from build123d import *

# Parameters (mm, degrees)
BOSS_EXTRUDE1_DEPTH                                 = 17.5
SKETCH2_W                                           = 25
SKETCH2_H                                           = 15
CUT_EXTRUDE1_DEPTH                                  = 47.435439053
M4_TAPPED_HOLE1_D                                   = 3.3
M4_TAPPED_HOLE1_DEPTH                               = 11.5
M4_TAPPED_HOLE1_TIP                                 = 0.991420021
SKETCH5_R                                           = 2
CUT_EXTRUDE2_DEPTH                                  = 56.452682532
FILLET1_R                                           = 2
SKETCH6_R                                           = 4
CUT_EXTRUDE3_DEPTH                                  = 3
CHAMFER1_SIZE                                       = 1
CBORE_FOR_M3_HEX_SOCKET_HEAD_CAP_SCREW1_D           = 3.4
CBORE_FOR_M3_HEX_SOCKET_HEAD_CAP_SCREW1_CBORE_D     = 6.5
CBORE_FOR_M3_HEX_SOCKET_HEAD_CAP_SCREW1_CBORE_DEPTH = 3.4


with BuildPart() as part:
    # Sketch1 → Boss-Extrude1 (new, symmetric)
    with BuildSketch(Plane.XY):
        Polygon((0, 0), (0, 35), (25, 35), (25, 27), (8, 27), (8, 0), align=None)
    extrude(amount=BOSS_EXTRUDE1_DEPTH, both=True)

    # Sketch2 → Cut-Extrude1 (cut, through all)
    with BuildSketch(Plane.ZY):
        with Locations((0, 17.5)):
            Rectangle(SKETCH2_W, SKETCH2_H)
    extrude(amount=-CUT_EXTRUDE1_DEPTH, mode=Mode.SUBTRACT)

    # M4 Tapped Hole1
    with Locations(Plane.ZY):
        with Locations((-12.5, 5), (12.5, 5)):
            Hole(M4_TAPPED_HOLE1_D / 2, depth=M4_TAPPED_HOLE1_DEPTH)
            with Locations((0, 0, -(M4_TAPPED_HOLE1_DEPTH + M4_TAPPED_HOLE1_TIP / 2))):  # 118° drill point
                Cone(0, M4_TAPPED_HOLE1_D / 2, M4_TAPPED_HOLE1_TIP, mode=Mode.SUBTRACT)

    # Sketch5 → Cut-Extrude2 (cut, through all)
    with BuildSketch(Plane.XY.offset(17.5)):
        with Locations((4, 17.5)):
            Circle(SKETCH5_R)
    extrude(amount=-CUT_EXTRUDE2_DEPTH, mode=Mode.SUBTRACT)

    # Fillet1
    fillet1_edges = [part.edges().sort_by_distance(p)[0] for p in [
        (4, 10, -12.5),
        (4, 25, -12.5),
        (4, 25, 12.5),
        (4, 10, 12.5),
    ]]
    fillet(fillet1_edges, radius=FILLET1_R)

    # Sketch6 → Cut-Extrude3 (cut)
    with BuildSketch(Plane.XZ.offset(-27)):
        with Locations((18, 0)):
            Circle(SKETCH6_R)
    extrude(amount=-CUT_EXTRUDE3_DEPTH, mode=Mode.SUBTRACT)

    # Chamfer1
    chamfer1_edges = [part.edges().sort_by_distance(p)[0] for p in [
        (0, 35, 0),
        (8, 27, 0),
        (25, 31, 17.5),
        (4, 0, 17.5),
        (25, 31, -17.5),
        (4, 0, -17.5),
    ]]
    chamfer(chamfer1_edges, length=CHAMFER1_SIZE)

    # CBORE for M3 Hex Socket Head Cap Screw1 (through all)
    with Locations(Plane(origin=(0, 35, 0), x_dir=(1, 0, 0), z_dir=(0, 1, 0))):
        with Locations((18, 0)):
            CounterBoreHole(CBORE_FOR_M3_HEX_SOCKET_HEAD_CAP_SCREW1_D / 2, CBORE_FOR_M3_HEX_SOCKET_HEAD_CAP_SCREW1_CBORE_D / 2, CBORE_FOR_M3_HEX_SOCKET_HEAD_CAP_SCREW1_CBORE_DEPTH)


solid = part.part
Check sheet for the modelled part. Datum: model origin and axes. Units: mm. A direction names the side the tool comes from. Round coordinates to 2 decimals unless told otherwise and drop trailing zeros. Loops run counter-clockwise (first coordinate to the right, second up) from the corner with the lowest first, then second, coordinate; pieces in that order, holes last. Notation, with made-up numbers: (2, 69) -> (55, 69) arc R25 cw to (55, 96) -> close; hole circle Ø4 at (-11, 52). An arc over 180 degrees is marked (long way). Put each result on its own line as item: value. Start each with the question number.
1. Section check A-A (y = 17.5). Enter the section's corners in (x, z).
2. Draft check along Z on faces 1 (the face through (7, 22, 17.5)), 2 (the face through (4, 0, 0)), 3 (the face through (4.056, 4.368, 10.976)). Enter one of: +Z half, -Z half, draft (parallel to the pull), parting line (faces both ways), or undercut.
3. Section check C-C (z = 0). Enter the section's corners in (x, y).
4. Section check B-B (x = 18). Enter the section's corners in (y, z), plus the area to 3 significant figures.
5. Scan lines: probe 1 along Z at (x, y) = (6.5, 23); probe 2 along Y at (x, z) = (4, 16); probe 3 along Y at (x, z) = (1, -3). Record each from-to range of solid material in increasing order.
6. Access from +Z, -Z, +X, -X, +Y, -Y to the whole of each face (thin tool, end or side, straight path). Record for faces 4 (the face through (4, 25, 0)), 5 (the face through (24.5, 31.1, 17)), 6 (the face through (4.1, 0.5, 17)), 7 (the face through (13.6, 27, 0.2)), 8 (the face through (18, 30, -2)).
7. Section check D-D (x = 4). Enter the section's corners in (y, z).
8. Gauge pin test, flat ends, axial feed: pin 1 (6.5 mm diameter, centred on x = 16, z = 0, fed in from -Y); pin 2 (5.5 mm diameter, centred on x = 18, z = 0, fed in from +Y); pin 3 (1.5 mm diameter, centred on x = 16, z = 0, fed in from -Y). Record the tip position at first contact, or that the pin passes through.
Findings:
1. outline: (0, -17.5) -> (2, -17.5) -> (2, -12.5) -> (0, -12.5) -> close; (0, 12.5) -> (2, 12.5) -> (2, 17.5) -> (0, 17.5) -> close; (6, -17.5) -> (8, -17.5) -> (8, -12.5) -> (6, -12.5) -> close; (6, 12.5) -> (8, 12.5) -> (8, 17.5) -> (6, 17.5) -> close
2. face 1: +Z half
2. face 2: draft
2. face 3: undercut
3. outline: (0, 0) -> (8, 0) -> (8, 10) -> (0, 10) -> close; (0, 25) -> (8, 25) -> (8, 26) -> (9, 27) -> (14, 27) -> (14, 30) -> (16.3, 30) -> (16.3, 31.6) -> (14.75, 31.6) -> (14.75, 35) -> (1, 35) -> (0, 34) -> close; (19.7, 30) -> (22, 30) -> (22, 27) -> (25, 27) -> (25, 35) -> (21.25, 35) -> (21.25, 31.6) -> (19.7, 31.6) -> close
4. outline: (27, -17.5) -> (35, -17.5) -> (35, -3.25) -> (31.6, -3.25) -> (31.6, -1.7) -> (30, -1.7) -> (30, -4) -> (27, -4) -> close; (27, 4) -> (30, 4) -> (30, 1.7) -> (31.6, 1.7) -> (31.6, 3.25) -> (35, 3.25) -> (35, 17.5) -> (27, 17.5) -> close
4. area: 228 mm^2
5. probe 1: z = -17.5 to -12.5, 12.5 to 17.5
5. probe 2: y = 0 to 15.5, 19.5 to 35
5. probe 3: y = 0 to 10, 25 to 35
6. face 4: +X, -X
6. face 5: +Z, +X, +Y, -Y
6. face 6: +Z, +X, -X, -Y
6. face 7: +Z, -Z, +X, -Y
6. face 8: -Y
7. outline: (0, -16.5) -> (1, -17.5) -> (15.5, -17.5) -> (15.5, -12.5) -> (12, -12.5) arc R2 cw to (10, -10.5) -> (10, 10.5) arc R2 cw to (12, 12.5) -> (15.5, 12.5) -> (15.5, 17.5) -> (1, 17.5) -> (0, 16.5) -> close; (19.5, -17.5) -> (35, -17.5) -> (35, 17.5) -> (19.5, 17.5) -> (19.5, 12.5) -> (23, 12.5) arc R2 cw to (25, 10.5) -> (25, -10.5) arc R2 cw to (23, -12.5) -> (19.5, -12.5) -> close; hole circle Ø3.3 at (5, -12.5); hole circle Ø3.3 at (5, 12.5)
8. pin 1: stops at y = 27
8. pin 2: stops at y = 31.6
8. pin 3: stops at y = 30
